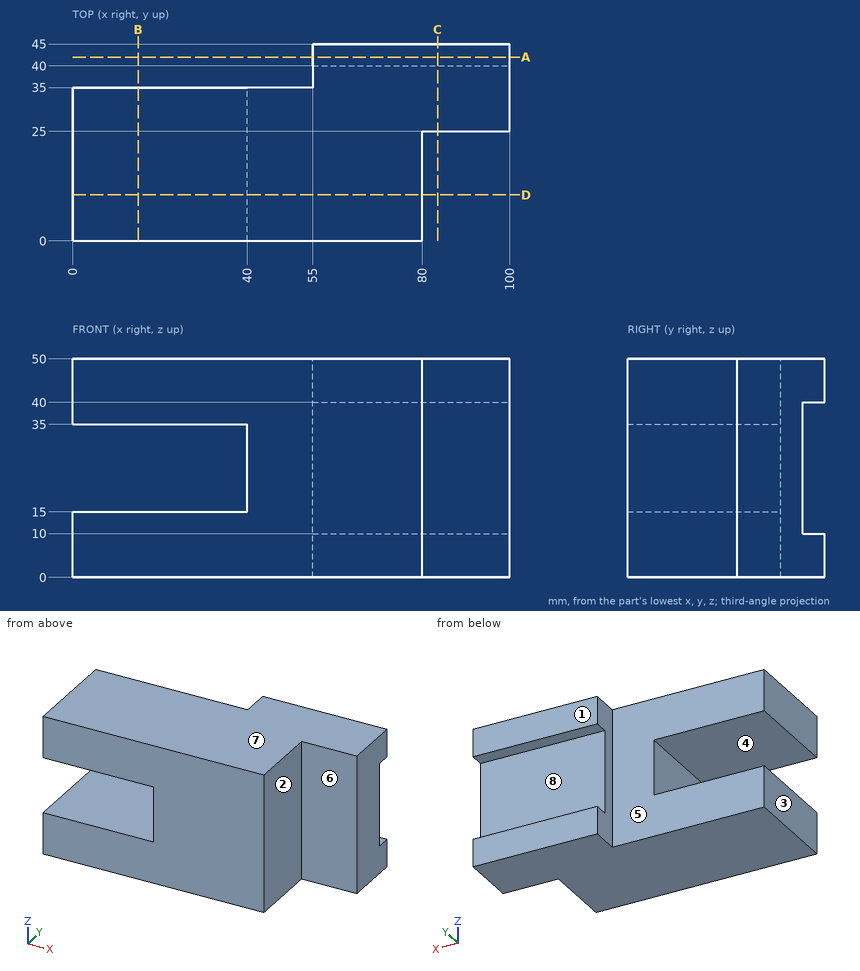
Verification items for this drawing (mm, ordinates from the low corner). A direction names the side the tool comes from. Give positions to 0.01 mm unless a question says otherwise; leave off trailing zeros. Write each loop counter-clockwise with the first axis right and the second up, starting at its lowest first coordinate (ties: lowest second). Pieces come first, ordered by that corner, then holes.
1) Section check B-B, the plane x = 15. Record the boundary of the cut face in (y, z), and give its area (3 significant figures).
2) Material ranges on L1, parallel to Z at x = 17, y = 3; L2, parallel to Z at x = 89, y = 41; L3, parallel to Y at x = 15, z = 13, recorded low to high.
3) Section check C-C, the plane x = 83.5. Record the boundary of the cut face in (y, z).
4) Access from +Z, -Z, +X, -X, +Y, -Y to the whole of each face (thin tool, end or side, straight path). Record for the marked faces 1, 2, 3, 4 and 5.
5) Release check for a two-part mould opening along Z. For the marked faces 6, 7 and 8 record: pulls with the +Z half, pulls with the -Z half, needs draft (parallel to the pull), parting line crosses it, or undercut.
6) Section check A-A, the plane y = 42. Record the boundary of the cut face in (x, z), and give its area (3 significant figures).
7) Gauge pin test, flat ends, axial feed: pin 1 (12 mm diameter, centred on y = 36.5, z = 22, fed in from -X); pin 2 (10 mm diameter, centred on x = 17, z = 44.5, fed in from +Y); pin 3 (2 mm diameter, centred on x = 76, z = 34.5, fed in from +Y); pin 4 (5 mm diameter, centred on x = 32.5, z = 19.5, fed in from -Y). Record the tip position at first contact, or that the pin passes through.
8) Section check D-D, the plane y = 10.5. Record the boundary of the cut face in (x, z).
Computed:
1. outline: (0, 0) - (35, 0) - (35, 15) - (0, 15) - close; (0, 35) - (35, 35) - (35, 50) - (0, 50) - close
1. area: 1,050 mm2
2. L1: z = 0 to 15, 35 to 50
2. L2: z = 0 to 10, 40 to 50
2. L3: y = 0 to 35
3. outline: (25, 0) - (45, 0) - (45, 10) - (40, 10) - (40, 40) - (45, 40) - (45, 50) - (25, 50) - close
4. face 1: +Z, -Z, +X, -X, +Y
4. face 2: +Z, -Z, +X, -Y
4. face 3: +Z, -Z, -X, +Y, -Y
4. face 4: -X, +Y, -Y
4. face 5: +Z, -Z, -X, +Y
5. face 6: needs draft
5. face 7: pulls with the +Z half
5. face 8: undercut
6. outline: (55, 0) - (100, 0) - (100, 10) - (55, 10) - close; (55, 40) - (100, 40) - (100, 50) - (55, 50) - close
6. area: 900 mm2
7. pin 1: stops at x = 40
7. pin 2: stops at y = 35
7. pin 3: stops at y = 40
7. pin 4: passes through
8. outline: (0, 0) - (80, 0) - (80, 50) - (0, 50) - (0, 35) - (40, 35) - (40, 15) - (0, 15) - close
